Check sheet for the modelled part. Datum: model origin and axes. Units: mm. Coordinates: 2 decimals unless noted, no trailing zeros. Write each loop counter-clockwise with the first axis right and the second up, starting at its lowest first coordinate (ties: lowest second). Pieces come first, ordered by that corner, then holes. Notation, with made-up numbers: (35.25, -36) -> (66.25, -36) arc R23 cw to (66.25, -26) -> close; hole circle Ø9 at (85, 7.5). An arc over 180 degrees is marked (long way). Put each result on its own line as item: value.
```python
from build123d import *

# Parameters (mm, degrees)
BOSS_EXTRUDE1_DEPTH = 190


with BuildPart() as part:
    # Sketch1 → Boss-Extrude1 (new, symmetric)
    with BuildSketch(Plane.XY):
        Polygon((0, 0), (0, 130), (-36, 130), (-36, 25.026825444), (-15, 0), align=None)
    extrude(amount=BOSS_EXTRUDE1_DEPTH, both=True)


solid = part.part
```
Q1. Cross-section at C-C (y = 18). Record the cut outline in (x, z), plus the area to 3 significant figures.
Recorded:
outline: (-30.1, -190) -> (0, -190) -> (0, 190) -> (-30.1, 190) -> close
area: 11,400 mm2
Q2. Depth check by flat-ended pin: P1, Ø8, axis at y = 99, z = 140, coming from the +X side; P2, Ø3, axis at x = -18.5, z = -111.5, coming from the -Y side. Enter the tip coordinate at first touch or a pass-through.
Recorded:
P1: stops at x = 0
P2: stops at y = 2.38
Q3. Cross-section at B-B (x = -26.5). Record the cut outline in (y, z).
Recorded:
outline: (13.71, -190) -> (130, -190) -> (130, 190) -> (13.71, 190) -> close
Q4. Mould release check, pull along Y, two halves, no side actions. Record for faces 1 (the flat face through (-18, 130, 3)), 2 (the flat face through (-8, 0, 3)), 3 (the flat face through (-18, 66, -190)): released by +Y, released by -Y, zero draft, split by the parting line, or undercut.
Recorded:
face 1: released by +Y
face 2: released by -Y
face 3: zero draft
Q5. Cross-section at A-A (z = -66.5). Record the cut outline in (x, y).
Recorded:
outline: (-36, 25.03) -> (-15, 0) -> (0, 0) -> (0, 130) -> (-36, 130) -> close
Q6. Material ranges on line 1 along Y through (x, z) = (-27, 4.5); line 2 along Y through (x, z) = (-26.5, 31.5); line 3 along X through (y, z) = (7, -163), recorded low to high.
Recorded:
line 1: y = 14.3 to 130
line 2: y = 13.71 to 130
line 3: x = -20.87 to 0
